from build123d import *

# Parameters (mm, degrees)
BOSS_EXTRUDE1_DEPTH  = 33.5
HOLE1_D              = 16
HOLE1_DEPTH          = 1.5
SKETCH4_R            = 8
SKETCH4_R_2          = 5.5
CUT_EXTRUDE1_DEPTH   = 5
HOLE2_D              = 4.134
HOLE2_DEPTH          = 6
HOLE2_CSINK_D        = 5
HOLE2_CSINK_ANGLE    = 90
LPATTERN1_COUNT      = 2
LPATTERN1_PITCH      = 20
LPATTERN2_COUNT      = 2
LPATTERN2_PITCH      = 20
LPATTERN2_COUNT_DIR2 = 2
LPATTERN2_PITCH_DIR2 = 20


with BuildPart() as part:
    # Sketch1 → Boss-Extrude1 (new body)
    with BuildSketch(Plane(origin=(0, 0, 0), x_dir=(0, 0, -1), z_dir=(1, 0, 0))):
        with BuildLine():
            Line((-12.278029158, -14.5), (-8, -14.5))
            Line((-8, -14.5), (-5.5, -12))
            Line((-5.5, -12), (5.5, -12))
            Line((5.5, -12), (8, -14.5))
            Line((8, -14.5), (12.278029158, -14.5))
            ThreePointArc((12.278029158, -14.5), (13.435028843, -13.435028843), (14.5, -12.278029158))
            Line((14.5, -12.278029158), (14.5, -8))
            Line((14.5, -8), (12, -5.5))
            Line((12, -5.5), (12, 5.5))
            Line((12, 5.5), (14.5, 8))
            Line((14.5, 8), (14.5, 12.278029158))
            ThreePointArc((14.5, 12.278029158), (13.435028843, 13.435028843), (12.278029158, 14.5))
            Line((12.278029158, 14.5), (8, 14.5))
            Line((8, 14.5), (6.5, 13))
            Line((6.5, 13), (5.401923789, 13))
            Line((5.401923789, 13), (5, 14.5))
            Line((5, 14.5), (-5, 14.5))
            Line((-5, 14.5), (-5.401923789, 13))
            Line((-5.401923789, 13), (-6.5, 13))
            Line((-6.5, 13), (-8, 14.5))
            Line((-8, 14.5), (-12.278029158, 14.5))
            ThreePointArc((-12.278029158, 14.5), (-13.435028843, 13.435028843), (-14.5, 12.278029158))
            Line((-14.5, 12.278029158), (-14.5, 8))
            Line((-14.5, 8), (-12, 5.5))
            Line((-12, 5.5), (-12, -5.5))
            Line((-12, -5.5), (-14.5, -8))
            Line((-14.5, -8), (-14.5, -12.278029158))
            ThreePointArc((-14.5, -12.278029158), (-13.435028843, -13.435028843), (-12.278029158, -14.5))
        make_face()
    extrude(amount=BOSS_EXTRUDE1_DEPTH)

    # Hole1
    with Locations(Plane(origin=(33.5, 0, 0), x_dir=(0, 0, -1), z_dir=(1, 0, 0))):
        with Locations((0, 0)):
            Hole(HOLE1_D / 2, depth=HOLE1_DEPTH)

    # Sketch4 → Cut-Extrude1 (cut)
    with BuildSketch(Plane(origin=(0, 0, 0), x_dir=(0, 0, -1), z_dir=(1, 0, 0))):
        Circle(SKETCH4_R)
        Circle(SKETCH4_R_2, mode=Mode.SUBTRACT)
    extrude(amount=CUT_EXTRUDE1_DEPTH, mode=Mode.SUBTRACT)

    # Sketch5 → Cut-Revolve1 (revolve, cut)
    with BuildSketch(Plane.XY, mode=Mode.PRIVATE) as cut_revolve1_sk:
        Polygon((0, 0), (0, 4), (10, 4), (10, 8), (30, 8), (30, 0), align=None)
    revolve(cut_revolve1_sk.sketch.rotate(Axis((30, 0, 0), (-1, 0, 0)), 270), axis=Axis((30, 0, 0), (-1, 0, 0)), mode=Mode.SUBTRACT)

    # Hole2
    with Locations(Plane(origin=(0, 14.5, 0), x_dir=(1, 0, 0), z_dir=(0, 1, 0))):
        with Locations((8, 0)):
            hole2 = CounterSinkHole(HOLE2_D / 2, HOLE2_CSINK_D / 2, depth=HOLE2_DEPTH, counter_sink_angle=HOLE2_CSINK_ANGLE)

    # LPattern1: Hole2 ×2
    with Locations(*[(i * LPATTERN1_PITCH, 0, 0) for i in range(1, LPATTERN1_COUNT)]):
        add(hole2, mode=Mode.SUBTRACT)

    # Sketch9 → Cut-Revolve2 (revolve, cut)
    with BuildSketch(Plane.XY.offset(10), mode=Mode.PRIVATE) as cut_revolve2_sk:
        Polygon((0, 10), (0, 13.25), (3.5, 13.25), (3.5, 11.75), (30, 11.75), (30, 13.25), (33.5, 13.25), (33.5, 10), align=None)
    cut_revolve2 = revolve(cut_revolve2_sk.sketch.rotate(Axis((33.5, 10, 10), (-1, 0, 0)), 270), axis=Axis((33.5, 10, 10), (-1, 0, 0)), mode=Mode.SUBTRACT)

    # LPattern2: Cut-Revolve2 2 × 2
    with Locations(*[(0, -j * LPATTERN2_PITCH_DIR2, -i * LPATTERN2_PITCH) for i in range(LPATTERN2_COUNT) for j in range(LPATTERN2_COUNT_DIR2) if (i, j) != (0, 0)]):
        add(cut_revolve2, mode=Mode.SUBTRACT)


solid = part.part
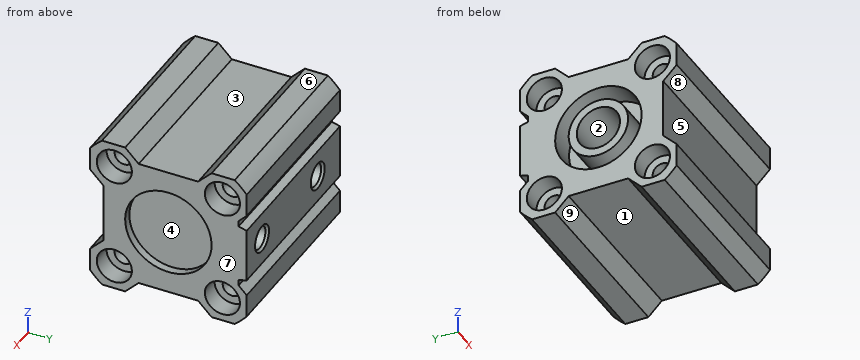
Verification items for the finished model (mm, model axes). Face numbers are marked on the shaded views. A direction names the side the tool comes from. Give positions to 0.01 mm unless a question says otherwise; leave off trailing zeros. Loops run counter-clockwise (first coordinate to the right, second up) from the corner with the lowest first, then second, coordinate; pieces in that order, holes last.
1) Draft check along Z on the marked faces 6, 7, 8 and 9. Enter one of: pulls with the +Z half, pulls with the -Z half, needs draft (parallel to the pull), parting line crosses it, or undercut.
2) Set-up check for the marked faces 1, 2, 3, 4 and 5: record each of +Z, -Z, +X, -X, +Y, -Y from which the full face is reachable in a straight line by a thin tool's end or side.
3) Sectioned sample at A-A, the plane z = 10. Enter the section's corners in (x, y), then the cut area to 3 significant figures.
4) Depth check by flat-ended pin: pin 1 Ø3 at (x, y) = (28.5, 0.5) entering from +Z; pin 2 Ø4.5 at (y, z) = (10, 10) entering from +X; pin 3 Ø3.5 at (x, z) = (8.5, 0) entering from +Y. Enter the tip coordinate at first touch or a pass-through.
5) Sectioned sample at B-B, the plane y = 10. Count the separate pieces of the cut face and the enclosed holes in it, then the cut area to 3 significant figures.
6) Thickness scan on line 1 along Y through (x, z) = (1.6, -10); line 2 along X through (y, z) = (-7.5, 1.5); line 3 along Y through (x, z) = (33.15, 0). Record the ranges inside material, lowest first.
Answers:
1. face 6: pulls with the +Z half
1. face 7: needs draft
1. face 8: undercut
1. face 9: pulls with the -Z half
2. face 1: -Z, +X, -X
2. face 2: -X
2. face 3: +Z, +X, -X
2. face 4: +X
2. face 5: +X, -X, -Y
3. outline: (0, -14.5) - (33.5, -14.5) - (33.5, -13.25) - (30, -13.25) - (30, -11.75) - (3.5, -11.75) - (3.5, -13.25) - (0, -13.25) - close; (0, -6.75) - (3.5, -6.75) - (3.5, -8.25) - (30, -8.25) - (30, -6.75) - (33.5, -6.75) - (33.5, 6.75) - (30, 6.75) - (30, 8.25) - (3.5, 8.25) - (3.5, 6.75) - (0, 6.75) - close; (0, 13.25) - (3.5, 13.25) - (3.5, 11.75) - (30, 11.75) - (30, 13.25) - (33.5, 13.25) - (33.5, 14.5) - (0, 14.5) - close
3. area: 695 mm2
4. pin 1: stops at z = 12
4. pin 2: stops at x = 30
4. pin 3: stops at y = 14.25
5. separate pieces: 3
5. enclosed holes: 2
5. area: 668 mm2
6. line 1: y = -14.5 to -13.25, -6.75 to 6.75, 13.25 to 14.5
6. line 2: x = 5 to 10, 30 to 32
6. line 3: y = -12 to -8, 8 to 14.5
